Read the model definition and answer for the solid it produces. Units are mm, in the model's axes. Face numbers are marked on the shaded views. A direction names the side the tool comes from. Coordinates: 2 decimals unless noted, no trailing zeros. Write each loop counter-clockwise with the first axis right and the second up, starting at its lowest first coordinate (ties: lowest second). Pieces come first, ordered by that corner, then holes.
1) The part is cut by section C-C (y = 17.75). Determine the outline of the cut face in (x, z).
2) The part is cut by section B-B (x = 0). Determine the outline of the cut face in (y, z), then the cut area to 3 significant figures.
3) Which of the six approach directions +Z, -Z, +X, -X, +Y, -Y give full straight-line access (tool end or side, diameter ignored) to the marked faces 4 and 5?
4) The part is cut by section A-A (z = 0). Determine the outline of the cut face in (x, y).
5) Determine the mould class of the marked faces 1, 2 and 3 for opening direction X: +X half, -X half, draft (parallel to the pull), parting line (faces both ways), or undercut.
6) Find the intervals of material crossed by line 1 (X direction, y = 11.5, z = 0); line 2 (X direction, y = 5.25, z = 0); line 3 (Y direction, x = 16, z = 7.5), in increasing order.
7) Each of these flat-tipped pins is pushed along its axis until it touches: pin 1 Ø5 at (x, y) = (-15, 7) entering from +Z; pin 2 Ø8 at (y, z) = (17.5, 11) entering from -X; pin 3 Ø2 at (x, y) = (7, 4.5) entering from -Z. Where does it stop, or does it pass through?
8) The part is cut by section D-D (y = 2.5). Determine the outline of the cut face in (x, z).
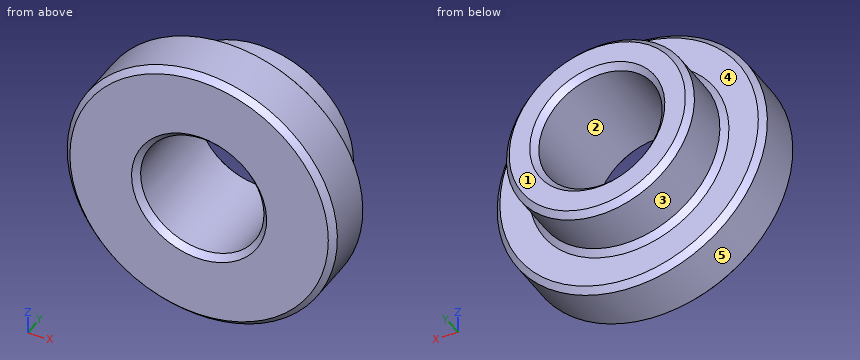
from build123d import *

# Parameters (mm, degrees)
SKETCH1_R           = 23
BOSS_EXTRUDE1_DEPTH = 10
SKETCH2_R           = 16
BOSS_EXTRUDE2_DEPTH = 10
SKETCH3_R           = 10.5
CUT_EXTRUDE1_DEPTH  = 20
CHAMFER1_SIZE       = 1
CHAMFER2_SIZE       = 1


with BuildPart() as part:
    # Sketch1 → Boss-Extrude1 (new body)
    with BuildSketch(Plane(origin=(0, 0, 0), x_dir=(1, 0, 0), z_dir=(0, 1, 0))):
        with Locations(Location((0, 0, 0), (0, 0, 270))):
            Circle(SKETCH1_R)
    extrude(amount=BOSS_EXTRUDE1_DEPTH)

    # Sketch2 → Boss-Extrude2 (add)
    with BuildSketch(Plane(origin=(0, 10, 0), x_dir=(1, 0, 0), z_dir=(0, 1, 0))):
        with Locations(Location((0, 0, 0), (0, 0, 270))):
            Circle(SKETCH2_R)
    extrude(amount=BOSS_EXTRUDE2_DEPTH)

    # Sketch3 → Cut-Extrude1 (cut)
    with BuildSketch(Plane(origin=(0, 20, 0), x_dir=(1, 0, 0), z_dir=(0, 1, 0))):
        with Locations(Location((0, 0, 0), (0, 0, 270))):
            Circle(SKETCH3_R)
    extrude(amount=-CUT_EXTRUDE1_DEPTH, mode=Mode.SUBTRACT)

    # Chamfer1
    chamfer1_edges = [part.edges().sort_by_distance(p)[0] for p in [
        (0, 20, -10.5),
        (0, 0, -23),
        (0, 10, -23),
        (0, 10, -16),
        (0, 20, -16),
    ]]
    chamfer(chamfer1_edges, length=CHAMFER1_SIZE)

    # Chamfer2
    chamfer2_edges = [part.edges().sort_by_distance(p)[0] for p in [
        (0, 0, -10.5),
    ]]
    chamfer(chamfer2_edges, length=CHAMFER2_SIZE)


solid = part.part
Reported:
1. outline: circle Ø32 at (0, 0); hole circle Ø21 at (0, 0)
2. outline: (0, -22) - (1, -23) - (9, -23) - (10, -22) - (10, -17) - (11, -16) - (19, -16) - (20, -15) - (20, -11.5) - (19, -10.5) - (1, -10.5) - (0, -11.5) - close; (0, 11.5) - (1, 10.5) - (19, 10.5) - (20, 11.5) - (20, 15) - (19, 16) - (11, 16) - (10, 17) - (10, 22) - (9, 23) - (1, 23) - (0, 22) - close
2. area: 356 mm2
3. face 4: +Y
3. face 5: +Y, -Y
4. outline: (-23, 1) - (-22, 0) - (-11.5, 0) - (-10.5, 1) - (-10.5, 19) - (-11.5, 20) - (-15, 20) - (-16, 19) - (-16, 11) - (-17, 10) - (-22, 10) - (-23, 9) - close; (10.5, 1) - (11.5, 0) - (22, 0) - (23, 1) - (23, 9) - (22, 10) - (17, 10) - (16, 11) - (16, 19) - (15, 20) - (11.5, 20) - (10.5, 19) - close
5. face 1: draft
5. face 2: undercut
5. face 3: parting line
6. line 1: x = -16 to -10.5, 10.5 to 16
6. line 2: x = -23 to -10.5, 10.5 to 23
6. line 3: y = 0 to 10
7. pin 1: stops at z = 19.31
7. pin 2: stops at x = -14.39
7. pin 3: stops at z = -22.2
8. outline: circle Ø46 at (0, 0); hole circle Ø21 at (0, 0)
